```python
from build123d import *

# Parameters (mm, degrees)
EXTRUDE_1_DEPTH              = 10
EXTRUDE_1_DEPTH_BACK         = 64
SKETCH_1_W                   = 70
SKETCH_1_H                   = 20
SKETCH_2_W                   = 70
SKETCH_2_H                   = 10
EXTRUDE_2_DEPTH              = 20
SKETCH_3_W                   = 70
SKETCH_3_H                   = 15
EXTRUDE_3_DEPTH              = 55
HOLE_WIZARD_M8_1_D           = 6.8
HOLE_WIZARD_M8_1_DEPTH       = 17.707073895
HOLE_WIZARD_M8_1_CSINK_D     = 8.05
HOLE_WIZARD_M8_1_CSINK_ANGLE = 90
HOLE_WIZARD_M8_1_TIP         = 2.042926105
HOLE_WIZARD_M6_1_D           = 5
HOLE_WIZARD_M6_1_DEPTH       = 13.497848452
HOLE_WIZARD_M6_1_CSINK_D     = 6.05
HOLE_WIZARD_M6_1_CSINK_ANGLE = 90
HOLE_WIZARD_M6_1_TIP         = 1.502151548


with BuildPart() as part:
    # 草图1 → 凸台-拉伸1 (new, two sides: drawn at the far end of the back side and taken through both)
    with BuildSketch(Plane.XY.offset(-EXTRUDE_1_DEPTH_BACK)):
        with Locations((0, 45)):
            Rectangle(SKETCH_1_W, SKETCH_1_H)
    extrude(amount=EXTRUDE_1_DEPTH + EXTRUDE_1_DEPTH_BACK)

    # 草图2 → 凸台-拉伸2 (add)
    with BuildSketch(Plane.XZ.offset(-35)):
        with Locations((0, 5)):
            Rectangle(SKETCH_2_W, SKETCH_2_H)
    extrude(amount=EXTRUDE_2_DEPTH)

    # 草图3 → 凸台-拉伸3 (add)
    with BuildSketch(Plane(origin=(0, 55, 0), x_dir=(1, 0, 0), z_dir=(0, 1, 0))):
        with Locations((0, 56.5)):
            Rectangle(SKETCH_3_W, SKETCH_3_H)
    extrude(amount=EXTRUDE_3_DEPTH)

    # M8 螺纹孔1
    with Locations(Plane.XY.offset(-49)):
        with Locations((25, 100), (25, 65), (-25, 65), (-25, 100)):
            CounterSinkHole(HOLE_WIZARD_M8_1_D / 2, HOLE_WIZARD_M8_1_CSINK_D / 2, depth=HOLE_WIZARD_M8_1_DEPTH, counter_sink_angle=HOLE_WIZARD_M8_1_CSINK_ANGLE)
            with Locations((0, 0, -(HOLE_WIZARD_M8_1_DEPTH + HOLE_WIZARD_M8_1_TIP / 2))):  # 118° drill point
                Cone(0, HOLE_WIZARD_M8_1_D / 2, HOLE_WIZARD_M8_1_TIP, mode=Mode.SUBTRACT)

    # M6 螺纹孔1
    with Locations(Plane.XY.offset(10)):
        with Locations((20, 25), (-20, 25)):
            CounterSinkHole(HOLE_WIZARD_M6_1_D / 2, HOLE_WIZARD_M6_1_CSINK_D / 2, depth=HOLE_WIZARD_M6_1_DEPTH, counter_sink_angle=HOLE_WIZARD_M6_1_CSINK_ANGLE)
            with Locations((0, 0, -(HOLE_WIZARD_M6_1_DEPTH + HOLE_WIZARD_M6_1_TIP / 2))):  # 118° drill point
                Cone(0, HOLE_WIZARD_M6_1_D / 2, HOLE_WIZARD_M6_1_TIP, mode=Mode.SUBTRACT)


solid = part.part
```
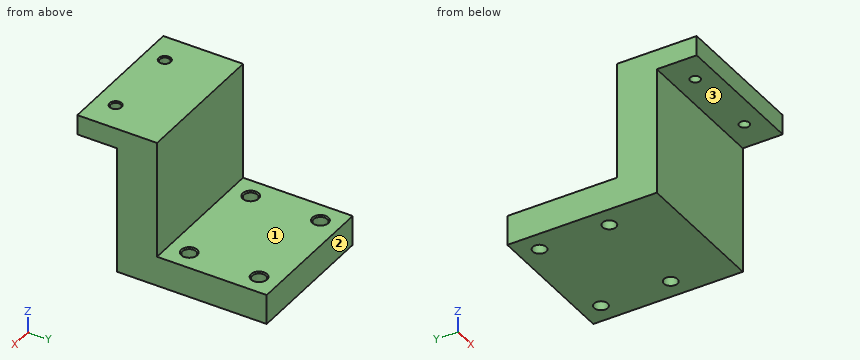
Model file for the job. Use its own axes, mm. Face numbers are marked on the shaded views. A direction names the side the tool comes from. Give positions to 0.01 mm unless a question says otherwise; leave off trailing zeros. Write each loop counter-clockwise with the first axis right and the second up, starting at its lowest first coordinate (ties: lowest second). Pieces come first, ordered by that corner, then holes. Notation, with made-up numbers: (-20, -28) - (32, -28) arc R23 cw to (32, -17) - close; hole circle Ø7 at (58.5, -11). An arc over 180 degrees is marked (long way). One line per question, with ' | ' between items. Start each with the question number.
(1) Slice it at D-D on x = -12.5. Write the cut outline in (y, z), plus the area to 4 significant figures.
(2) Wall check: line 1 along Y through (x, z) = (-25, -52); line 2 along X through (y, z) = (65, -57); line 3 along X through (y, z) = (25, 5.5). Give the ranges that are in metal, low to high. Write a range as from..to.
(3) Slice it at B-B on z = -57. Write the cut outline in (x, y).
(4) Slice it at C-C on x = 25. Write the cut outline in (y, z) (3 decimals), plus the area to 3 significant figures.
(5) Slice it at A-A on y = 65. Write the cut outline in (x, z) (3 decimals).
(6) Pin check, flat tips, straight feed: P1, Ø6, axis at x = 20, y = 25, coming from the +Z side (3 decimals); P2, Ø16, axis at x = 9.5, y = 25.5, coming from the -Z side; P3, Ø2, axis at x = -6, y = 98.5, coming from the +Z side; P4, Ø5.5, axis at x = 25, y = 65, coming from the +Z side. Stop position of each tip, or through.
(7) 3-axis set-ups, long thin cutter, end or side, ignore diameter. For the marked faces 1, 2 and 3: which of +Z, -Z, +X, -X, +Y, -Y reach the whole face in a straight line?
Results below:
1) outline: (15, 0) - (35, 0) - (35, -64) - (110, -64) - (110, -49) - (55, -49) - (55, 10) - (15, 10) - close | area: 2,505 mm^2
2) line 1: 35..61.6, 68.4..96.6, 103.4..110 | line 2: -35..-28.4, -21.6..21.6, 28.4..35 | line 3: -35..-22.5, -17.5..17.5, 22.5..35
3) outline: (-35, 35) - (35, 35) - (35, 110) - (-35, 110) - close; hole circle Ø6.8 at (-25, 65); hole circle Ø6.8 at (-25, 100); hole circle Ø6.8 at (25, 65); hole circle Ø6.8 at (25, 100)
4) outline: (15, 0) - (35, 0) - (35, -64) - (61.6, -64) - (61.6, -49.625) - (60.975, -49) - (55, -49) - (55, 10) - (15, 10) - close; (68.4, -64) - (96.6, -64) - (96.6, -49.625) - (95.975, -49) - (69.025, -49) - (68.4, -49.625) - close; (103.4, -64) - (110, -64) - (110, -49) - (104.025, -49) - (103.4, -49.625) - close | area: 2,300 mm^2
5) outline: (-35, -64) - (-28.4, -64) - (-28.4, -49.625) - (-29.025, -49) - (-35, -49) - close; (-21.6, -64) - (21.6, -64) - (21.6, -49.625) - (20.975, -49) - (-20.975, -49) - (-21.6, -49.625) - close; (28.4, -64) - (35, -64) - (35, -49) - (29.025, -49) - (28.4, -49.625) - close
6) P1: z = 9.975 | P2: z = 0 | P3: z = -49 | P4: through
7) face 1: +Z, +X, -X, +Y | face 2: +Z, -Z, +X, -X, +Y | face 3: -Z, +X, -X, -Y
